For this review, take the finished solid that the model builds, in its own axes (mm). A direction names the side the tool comes from. Give positions to 0.01 mm unless a question says otherwise; leave off trailing zeros. Write each loop counter-clockwise with the first axis right and the second up, starting at its lowest first coordinate (ties: lowest second). Pieces come first, ordered by that corner, then holes. Notation, with made-up numbers: M 59,17 L 83,17 A13 cw 83,25 Z; hole C 84.25,-2 d1. An arc over 180 degrees is marked long. Use one line per item in the form item = value. Start each with the question number.
Q1. For probe 1 along Y at (x, z) = (4.25, -2.75); probe 2 along Z at (x, y) = (1.5, -14.5); probe 3 along X at (y, z) = (-16.5, 3.5), list the stretches that pass through material, from the lowest coordinate up. Write a range as [from, to].
Q2. Consider section A-A on y = 18. Write out the cut boundary in (x, z).
Q3. Mouldability with a two-part tool opening along Z and no side actions: class faces 3 (the cylindrical face through (2.44, -15.56, 0.54)), 4 (the cylindrical face through (-3.905, 21.472, -0.867)), 5 (the flat face through (-2.41, 0.27, 4.11)) as released by +Z, released by -Z, zero draft, split by the parting line, or undercut.
Q4. Tool access review of faces 1 (the flat face through (2, 19.5, 4)), 2 (the flat face through (2.41, 0.27, -4.11)): name each direction out of +Z, -Z, +X, -X, +Y, -Y from which nothing blocks a thin tool from reaching the whole face with its end or side.
Q5. Clearance check with flat-ended pins moving along their axes: pin 1 Ø1 at (y, z) = (17, -4) entering from -X; pin 2 Ø4 at (y, z) = (0.5, -4) entering from +X; pin 3 Ø1 at (x, y) = (-2, 15.5) entering from -Z. State where each tip first meets the part, or that it passes through.
```python
from build123d import *

# Parameters (mm, degrees)
BOSS_EXTRUDE1_DEPTH = 19.5
SKETCH3_R           = 4
BOSS_EXTRUDE2_DEPTH = 5
CHAMFER1_SIZE       = 1


with BuildPart() as part:
    # Sketch1 → Boss-Extrude1 (new, symmetric)
    with BuildSketch(Plane(origin=(0, 0, 0), x_dir=(1, 0, 0), z_dir=(0, 1, 0))):
        Polygon((0, 5.5), (-4.763139721, 2.75), (-4.763139721, -2.75), (0, -5.5), (4.763139721, -2.75), (4.763139721, 2.75), align=None)
    extrude(amount=BOSS_EXTRUDE1_DEPTH, both=True)

    # Sketch3 → Boss-Extrude2 (add)
    with BuildSketch(Plane(origin=(0, 19.5, 0), x_dir=(1, 0, 0), z_dir=(0, 1, 0))):
        with Locations(Location((0, 0, 0), (0, 0, 270))):
            Circle(SKETCH3_R)
    extrude(amount=BOSS_EXTRUDE2_DEPTH)

    # Chamfer1
    chamfer1_edges = [part.edges().sort_by_distance(p)[0] for p in [
        (0, 24.5, -4),
    ]]
    chamfer(chamfer1_edges, length=CHAMFER1_SIZE)

    # Sketch6 → M6x1.0 Tapped Hole2 (revolve, cut)
    with BuildSketch(Plane(origin=(-4.548e-06, -19.5, 2.5825e-05), x_dir=(0, 0, -1), z_dir=(1, 0, 0))):
        Polygon((0, 0), (0, 9.502151548), (2.5, 8), (2.5, 0), align=None)
    revolve(axis=Axis((-4.548e-06, -25.85, 2.5825e-05), (0, 1, 0)), mode=Mode.SUBTRACT)


solid = part.part
```
Working result:
q1.probe_1 = [-19.5, 19.5]
q1.probe_2 = [-4.63, -2], [2, 4.63]
q1.probe_3 = [-3.46, 3.46]
q2.outline = M -4.76,-2.75 L 0,-5.5 L 4.76,-2.75 L 4.76,2.75 L 0,5.5 L -4.76,2.75 Z
q3.face_3 = undercut
q3.face_4 = split by the parting line
q3.face_5 = released by +Z
q4.face_1 = +Y
q4.face_2 = -Z, +X, +Y, -Y
q5.pin_1 = -3.46
q5.pin_2 = 4.76
q5.pin_3 = -4.63
